Verification items for the finished model (mm, model axes). Round coordinates to 2 decimals unless told otherwise and drop trailing zeros. Write each loop counter-clockwise with the first axis right and the second up, starting at its lowest first coordinate (ties: lowest second). Pieces come first, ordered by that corner, then holes. Notation, with made-up numbers: (19, -7.5) -> (68, -7.5) arc R11 ccw to (68, 13.5) -> close; hole circle Ø2 at (-23, 67). An arc over 180 degrees is marked (long way). Answer as a JSON object with one key per item and string values. Group by question number.
(1) Draft check along X on faces 1 (the face through (-2.4, 7.9, 4.5)), 2 (the face through (-5, 16, -4)), 3 (the face through (20, 8, 0)). Enter one of: released by +X, released by -X, zero draft, split by the parting line, or undercut.
(2) Sectioned sample at B-B on z = 0. Record the cut outline in (x, y), and give its area (3 significant figures).
(3) Sectioned sample at C-C on y = 11. Record the cut outline in (x, z).
(4) Scan lines: L1, parallel to Z at x = 0, y = 9.5; L2, parallel to X at y = 5.25, z = -1; L3, parallel to X at y = 1.5, z = -3.25. Record each from-to range of solid material in increasing order. Write a range as from..to.
(5) Sectioned sample at A-A on x = -4.5. Record the cut outline in (y, z), and give its area (3 significant figures).
```python
from build123d import *

# Parameters (mm, degrees)
SKETCH1_W           = 40
SKETCH1_H           = 30
BOSS_EXTRUDE1_DEPTH = 16
M12_TAPPED_HOLE1_D  = 10.2


with BuildPart() as part:
    # Sketch1 → Boss-Extrude1 (new body)
    with BuildSketch(Plane(origin=(0, 0, 0), x_dir=(1, 0, 0), z_dir=(0, 1, 0))):
        Rectangle(SKETCH1_W, SKETCH1_H)
    extrude(amount=BOSS_EXTRUDE1_DEPTH)

    # M12 Tapped Hole1 (through all)
    with Locations(Plane(origin=(0, 16, 0), x_dir=(1, 0, 0), z_dir=(0, 1, 0))):
        with Locations((0, 0)):
            Hole(M12_TAPPED_HOLE1_D / 2)


solid = part.part
```
Computed values:
{
 "1": {"face 1": "undercut", "face 2": "zero draft", "face 3": "released by +X"},
 "2": {"outline": "(-20, 0) -> (-5.1, 0) -> (-5.1, 16) -> (-20, 16) -> close; (5.1, 0) -> (20, 0) -> (20, 16) -> (5.1, 16) -> close", "area": "477 mm2"},
 "3": {"outline": "(-20, -15) -> (20, -15) -> (20, 15) -> (-20, 15) -> close; hole circle Ø10.2 at (0, 0)"},
 "4": {"L1": "-15..-5.1, 5.1..15", "L2": "-20..-5, 5..20", "L3": "-20..-3.93, 3.93..20"},
 "5": {"outline": "(0, -15) -> (16, -15) -> (16, -2.4) -> (0, -2.4) -> close; (0, 2.4) -> (16, 2.4) -> (16, 15) -> (0, 15) -> close", "area": "403 mm2"}
}
